The model under review builds one solid part; all positions refer to its coordinate system, in mm. Give positions to 0.01 mm unless a question says otherwise; leave off trailing zeros. Loops run counter-clockwise (first coordinate to the right, second up) from the corner with the lowest first, then second, coordinate; pieces in that order, holes last. Notation, with made-up numbers: (84.25, -11.5) - (116.25, -11.5) arc R20 cw to (116.25, 26.5) - close; hole circle Ø9 at (20.5, 21). An arc over 180 degrees is marked (long way). Return JSON: item names as keys, results as strings. Group by question number.
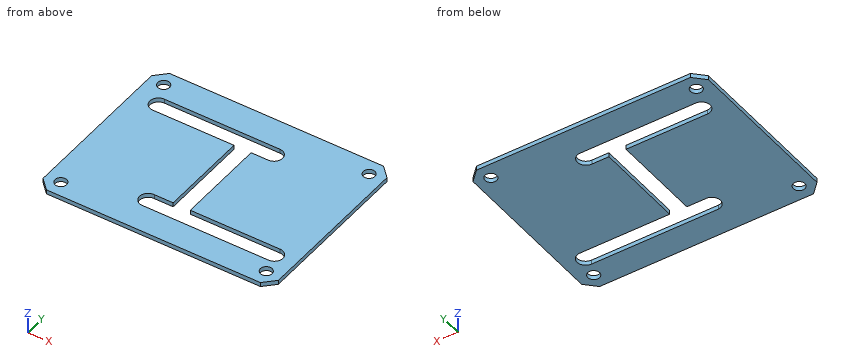
from build123d import *

# Parameters (mm, degrees)
EXTRUDE_1_DEPTH     = 2
CUT_EXTRUDE_1_DEPTH = 2
SKETCH_3_R          = 2.75
CUT_EXTRUDE_2_DEPTH = 2


with BuildPart() as part:
    # 草图1 → 凸台-拉伸1 (new body)
    with BuildSketch(Plane.XY):
        Polygon((357, 44.4274829), (457, 44.4274829), (462, 49.4274829), (462, 124.4274829), (457, 129.4274829), (357, 129.4274829), (352, 124.4274829), (352, 49.4274829), align=None)
    extrude(amount=EXTRUDE_1_DEPTH)

    # 草图2 → 切除-拉伸1 (cut)
    with BuildSketch(Plane.XY.offset(2)):
        with BuildLine():
            Line((452, 57.4274829), (392.718534883, 57.4274829))
            ThreePointArc((392.718534883, 57.4274829), (389, 61.708948017), (393.281465117, 65.4274829))
            Line((393.281465117, 65.4274829), (402, 65.4274829))
            Line((402, 65.4274829), (402, 107.4274829))
            Line((402, 107.4274829), (364, 107.4274829))
            ThreePointArc((364, 107.4274829), (360, 111.4274829), (364, 115.4274829))
            Line((364, 115.4274829), (418, 115.4274829))
            ThreePointArc((418, 115.4274829), (422, 111.4274829), (418, 107.4274829))
            Line((418, 107.4274829), (410, 107.4274829))
            Line((410, 107.4274829), (410, 65.4274829))
            Line((410, 65.4274829), (452, 65.4274829))
            ThreePointArc((452, 65.4274829), (456, 61.4274829), (452, 57.4274829))
        make_face()
    extrude(amount=-CUT_EXTRUDE_1_DEPTH, mode=Mode.SUBTRACT)

    # 草图3 → 切除-拉伸2 (cut)
    with BuildSketch(Plane.XY.offset(2)):
        with Locations((455, 51.4274829)):
            Circle(SKETCH_3_R)
        with Locations((359, 51.4274829)):
            Circle(SKETCH_3_R)
        with Locations((455, 122.4274829)):
            Circle(SKETCH_3_R)
        with Locations((359, 122.4274829)):
            Circle(SKETCH_3_R)
    extrude(amount=-CUT_EXTRUDE_2_DEPTH, mode=Mode.SUBTRACT)


solid = part.part
Item 1: Take a section at A-A (x = 449). State the section outline as (y, z) points.
Item 2: For P1, Ø3.5, axis at x = 359, y = 122.43, coming from the +Z side, flat-tipped, find the tip position at first contact; note if it passes through.
Item 3: Take a section at C-C (z = 1.35). State the section outline as (x, y) points, then the cut area to 3 significant figures.
Item 4: Take a section at B-B (y = 88.5). State the section outline as (x, z) points.
Item 5: For L1, parallel to Y at x = 415, z = 0.1; L2, parallel to Y at x = 359, z = 0.4; L3, parallel to Y at x = 428, z = 1.05, list the stretches that pass through material, from the lowest coordinate up. Write a range as from..to.
Check sheet entries:
{
 "1": {"outline": "(44.43, 0) - (57.43, 0) - (57.43, 2) - (44.43, 2) - close; (65.43, 0) - (129.43, 0) - (129.43, 2) - (65.43, 2) - close"},
 "2": {"P1": "passes through"},
 "3": {"outline": "(352, 49.43) - (357, 44.43) - (457, 44.43) - (462, 49.43) - (462, 124.43) - (457, 129.43) - (357, 129.43) - (352, 124.43) - close; hole circle Ø5.5 at (359, 51.43); hole circle Ø5.5 at (359, 122.43); hole (364, 107.43) - (402, 107.43) - (402, 65.43) - (393.28, 65.43) arc R4.01 ccw to (392.72, 57.43) - (452, 57.43) arc R4 ccw to (452, 65.43) - (410, 65.43) - (410, 107.43) - (418, 107.43) arc R4 ccw to (418, 115.43) - (364, 115.43) arc R4 ccw to start; hole circle Ø5.5 at (455, 51.43); hole circle Ø5.5 at (455, 122.43)", "area": "7,860 mm^2"},
 "4": {"outline": "(352, 0) - (402, 0) - (402, 2) - (352, 2) - close; (410, 0) - (462, 0) - (462, 2) - (410, 2) - close"},
 "5": {"L1": "y = 44.43..57.43, 65.43..107.43, 115.43..129.43", "L2": "y = 44.43..48.68, 54.18..119.68, 125.18..129.43", "L3": "y = 44.43..57.43, 65.43..129.43"}
}
